from build123d import *

# Parameters (mm, degrees)
SKETCH2_R          = 3.25
CUT_EXTRUDE1_DEPTH = 55.074023338


with BuildPart() as part:
    # Sketch1 → Revolve1 (revolve)
    with BuildSketch(Plane.XY, mode=Mode.PRIVATE) as revolve1_sk:
        Polygon((0, 0), (0, 38), (-6, 38), (-6, 33), (-4, 33), (-4, 0), align=None)
    revolve(revolve1_sk.sketch.rotate(Axis((0, 0, 0), (-1, 0, 0)), 90), axis=Axis((0, 0, 0), (-1, 0, 0)))

    # Sketch2 → Cut-Extrude1 (cut, through all)
    with BuildSketch(Plane(origin=(0, 0, 0), x_dir=(0, 0, -1), z_dir=(1, 0, 0))):
        with Locations((0, 15)):
            Circle(SKETCH2_R)
        with Locations((0, -15)):
            Circle(SKETCH2_R)
    extrude(amount=-CUT_EXTRUDE1_DEPTH, mode=Mode.SUBTRACT)


solid = part.part
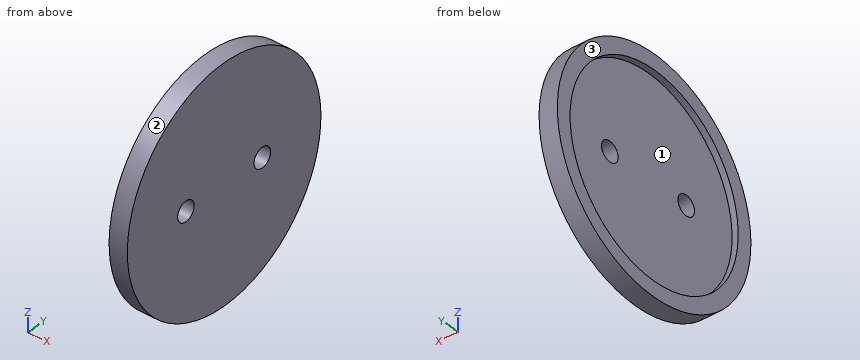
The model under review builds one solid part; all positions refer to its coordinate system, in mm. Face numbers are marked on the shaded views. Give positions to 0.01 mm unless a question says otherwise; leave off trailing zeros. Write each loop counter-clockwise with the first axis right and the second up, starting at its lowest first coordinate (ties: lowest second). Pieces come first, ordered by that corner, then holes.
1. Draft analysis for pull direction Z (two halves, no side actions). For the marked faces 1, 2 and 3, state which applies: +Z half, -Z half, draft (parallel to the pull), parting line (faces both ways), or undercut.
2. For P1, Ø1.5, axis at x = -1.5, y = 11, coming from the +Z side; P2, Ø1, axis at x = -1, z = -23.5, coming from the +Y side, all flat-tipped, find the tip position at first contact; note any pin that passes through.
3. Add section C-C, the plane y = -15. Write out the cut boundary in (x, z).
4. Add section D-D, the plane x = -4.9. Write out the cut boundary in (y, z).
5. Add section A-A, the plane z = 0. Write out the cut boundary in (x, y), plus the area to 3 significant figures.
6. Wall thickness on L1, parallel to Y at x = -5.1, z = 0; L2, parallel to Y at x = -3.2, z = 3; L3, parallel to Y at x = -3.45, z = -1: over which ranges is each line inside the solid? List them lowest first.
7. Add section B-B, the plane y = 0. Write out the cut boundary in (x, z).
Worked answers:
1. face 1: undercut
1. face 2: parting line
1. face 3: draft
2. P1: stops at z = 36.59
2. P2: stops at y = 30.25
3. outline: (-6, -34.91) - (0, -34.91) - (0, -3.25) - (-4, -3.25) - (-4, -29.39) - (-6, -29.39) - close; (-6, 29.39) - (-4, 29.39) - (-4, 3.25) - (0, 3.25) - (0, 34.91) - (-6, 34.91) - close
4. outline: circle Ø76 at (0, 0); hole circle Ø66 at (0, 0)
5. outline: (-6, -38) - (0, -38) - (0, -18.25) - (-4, -18.25) - (-4, -33) - (-6, -33) - close; (-6, 33) - (-4, 33) - (-4, 18.25) - (0, 18.25) - (0, 38) - (-6, 38) - close; (-4, -11.75) - (0, -11.75) - (0, 11.75) - (-4, 11.75) - close
5. area: 272 mm2
6. L1: y = -38 to -33, 33 to 38
6. L2: y = -37.88 to -16.25, -13.75 to 13.75, 16.25 to 37.88
6. L3: y = -37.99 to -18.09, -11.91 to 11.91, 18.09 to 37.99
7. outline: (-6, -38) - (0, -38) - (0, 38) - (-6, 38) - (-6, 33) - (-4, 33) - (-4, -33) - (-6, -33) - close
